The listing builds one solid part. Answer for the finished solid, in the listing's coordinates (mm). A direction names the side the tool comes from. Give positions to 0.01 mm unless a question says otherwise; leave off trailing zeros. Order: outer loops, then holes, each group sorted by start corner. A loop starts at its lowest first (then second) coordinate and runs counter-clockwise, first axis right, second up. Notation, with made-up numbers: M 33.5,77.5 L 79.5,77.5 A14 ccw 79.5,101.5 Z; hole C 20.25,29 d6. An arc over 180 degrees is marked long. Answer as a JSON object with one key per item and string values. Group by question number.
```python
from build123d import *

# Parameters (mm, degrees)
SKETCH_1_R                   = 56
EXTRUDE_1_DEPTH              = 10
SKETCH_2_R                   = 15
EXTRUDE_2_DEPTH              = 25
M20X1_5_1_D                  = 18.5
M20X1_5_1_DEPTH              = 44.5
M20X1_5_1_TIP                = 5.557960726
HOLE_WIZARD_M6_1_D           = 6.6
HOLE_WIZARD_M6_1_CSINK_D     = 13.44
HOLE_WIZARD_M6_1_CSINK_ANGLE = 90
SKETCH_12_OUTSIDE_W          = 146.442
SKETCH_12_OUTSIDE_H          = 146.442
SKETCH_12_OUTSIDE_W_2        = 136.125327254
SKETCH_12_OUTSIDE_H_2        = 80
CUT_EXTRUDE_1_DEPTH          = 25
SKETCH_13_W                  = 2
SKETCH_13_H                  = 2.5
CHAMFER_7_SIZE               = 0.5
SKETCH_14_R                  = 15
CUT_EXTRUDE_2_DEPTH          = 5


with BuildPart() as part:
    # 草图1 → 凸台-拉伸1 (new body)
    with BuildSketch(Plane(origin=(0, 0, 0), x_dir=(1, 0, 0), z_dir=(0, 1, 0))):
        with Locations(Location((0, 0, 0), (0, 0, 270))):
            Circle(SKETCH_1_R)
    extrude(amount=EXTRUDE_1_DEPTH)

    # 草图2 → 凸台-拉伸2 (add)
    with BuildSketch(Plane(origin=(0, 10, 0), x_dir=(1, 0, 0), z_dir=(0, 1, 0))):
        with Locations(Location((0, 0, 0), (0, 0, 270))):
            Circle(SKETCH_2_R)
    extrude(amount=EXTRUDE_2_DEPTH)

    # M20x1.5 螺纹孔1
    with Locations(Plane(origin=(0, 35, 0), x_dir=(1, 0, 0), z_dir=(0, 1, 0))):
        with Locations((0, 0)):
            Hole(M20X1_5_1_D / 2, depth=M20X1_5_1_DEPTH)
            with Locations((0, 0, -(M20X1_5_1_DEPTH + M20X1_5_1_TIP / 2))):  # 118° drill point
                Cone(0, M20X1_5_1_D / 2, M20X1_5_1_TIP, mode=Mode.SUBTRACT)

    # M6 六角凹锥坑螺钉的锥形沉头孔1 (through all)
    with Locations(Plane(origin=(0, 10, 0), x_dir=(1, 0, 0), z_dir=(0, 1, 0))):
        with Locations((44.346217561, -18.368804754), (-44.346217561, 18.368804754), (-44.346217561, -18.368804754), (44.346217561, 18.368804754)):
            CounterSinkHole(HOLE_WIZARD_M6_1_D / 2, HOLE_WIZARD_M6_1_CSINK_D / 2, counter_sink_angle=HOLE_WIZARD_M6_1_CSINK_ANGLE)

    # 草图12 outside → 切除-拉伸1 (cut)
    with BuildSketch(Plane(origin=(0, 10, 0), x_dir=(1, 0, 0), z_dir=(0, 1, 0))):
        Rectangle(SKETCH_12_OUTSIDE_W, SKETCH_12_OUTSIDE_H)
        Rectangle(SKETCH_12_OUTSIDE_W_2, SKETCH_12_OUTSIDE_H_2, mode=Mode.SUBTRACT)
    extrude(amount=-CUT_EXTRUDE_1_DEPTH, mode=Mode.SUBTRACT)

    # 草图13 → 切除-旋转1 (revolve, cut)
    with BuildSketch(Plane.XY, mode=Mode.PRIVATE) as cut_revolve_1_sk:
        with Locations((-14, 11.25)):
            Rectangle(SKETCH_13_W, SKETCH_13_H)
    revolve(cut_revolve_1_sk.sketch.rotate(Axis((0, -2.79729943, 0), (0, 1, 0)), 270), axis=Axis((0, -2.79729943, 0), (0, 1, 0)), mode=Mode.SUBTRACT)

    # 倒角7
    chamfer_7_edges = [part.edges().sort_by_distance(p)[0] for p in [
        (56, 0, 0),
        (56, 10, 0),
        (-56, 0, 0),
        (0, 0, -40),
        (0, 0, 40),
        (-56, 10, 0),
        (0, 10, 40),
        (0, 10, -40),
        (0, 35, -15),
    ]]
    chamfer(chamfer_7_edges, length=CHAMFER_7_SIZE)

    # 草图14 → 切除-拉伸2 (cut)
    with BuildSketch(Plane.XZ):
        with Locations(Location((0, 0, 0), (0, 0, 270))):
            Circle(SKETCH_14_R)
    extrude(amount=-CUT_EXTRUDE_2_DEPTH, mode=Mode.SUBTRACT)


solid = part.part
```
Item 1: A tool of negligible diameter and unlimited length cuts with its end or side. For faces 4 (the conical face through (-55.632, 9.865, -0.62)), 5 (the cylindrical face through (0.66, 2.465, 14.985)), 6 (the flat face through (-13.4, 12.5, 0.1)), from which of +Z, -Z, +X, -X, +Y, -Y can it reach the whole face along a straight path? Write none if from no direction.
Item 2: Consider probe 1 along Z at (x, y) = (-45, 3); probe 2 along Y at (x, z) = (-36, -26); probe 3 along Z at (x, y) = (1.5, 21). Determine where each line is inside the solid, lowest interval first. Write a range as from..to.
Item 3: Section D-D (y = 23.5) is taken. Determine the outline of the cut face in (x, z), and give its area (3 significant figures).
Item 4: Section B-B (z = 0) is taken. Determine the outline of the cut face in (x, y), and give its area (3 significant figures).
Item 5: Flat-ended cylindrical pins translate along their axes: P1, Ø6, axis at x = 7, y = 24, coming from the -Z side; P2, Ø4, axis at x = -44.35, z = -18.37, coming from the +Y side (3 decimals); P3, Ø6, axis at x = -42, y = 12, coming from the +Z side; P4, Ø8.5, axis at x = 44.35, z = -18.37, coming from the +Y side. Find the tip coordinate at first contact, or state that the pin passes through.
Item 6: Determine the mould class of faces 1 (the cylindrical face through (55.997, 4.937, 0.624)), 2 (the conical face through (41.04, 6.746, 17.328)), 3 (the flat face through (13, 0, 8)) for opening direction Z: released by +Z, released by -Z, zero draft, split by the parting line, or undercut.
Item 7: Section C-C (x = -30) is taken. Determine the outline of the cut face in (y, z).
Item 8: Section A-A (x = 0) is taken. Determine the outline of the cut face in (y, z).
Values found:
{
 "1": {"face 4": "-X, +Y", "face 5": "-Y", "face 6": "none"},
 "2": {"probe 1": "z = -33.33..-21.6, -15.13..15.13, 21.6..33.33", "probe 2": "y = 0..10", "probe 3": "z = -14.92..-9.13, 9.13..14.92"},
 "3": {"outline": "C 0,0 d30; hole C 0,0 d18.5", "area": "438 mm^2"},
 "4": {"outline": "M -56,0.5 L -55.5,0 L -15,0 L -15,5 L -9.25,5 L -9.25,35 L -14.5,35 L -15,34.5 L -15,12.5 L -13,12.5 L -13,10 L -55.5,10 L -56,9.5 Z; M 9.25,5 L 15,5 L 15,0 L 55.5,0 L 56,0.5 L 56,9.5 L 55.5,10 L 13,10 L 13,12.5 L 15,12.5 L 15,34.5 L 14.5,35 L 9.25,35 Z", "area": "1,150 mm^2"},
 "5": {"P1": "stops at z = -14.46", "P2": "passes through", "P3": "stops at z = 38.84", "P4": "stops at y = 7.53"},
 "6": {"face 1": "split by the parting line", "face 2": "undercut", "face 3": "zero draft"},
 "7": {"outline": "M 0,-39.5 L 0.5,-40 L 9.5,-40 L 10,-39.5 L 10,39.5 L 9.5,40 L 0.5,40 L 0,39.5 Z"},
 "8": {"outline": "M 0,-39.5 L 0.5,-40 L 9.5,-40 L 10,-39.5 L 10,-13 L 12.5,-13 L 12.5,-15 L 34.5,-15 L 35,-14.5 L 35,-9.25 L 5,-9.25 L 5,-15 L 0,-15 Z; M 0,15 L 5,15 L 5,9.25 L 35,9.25 L 35,14.5 L 34.5,15 L 12.5,15 L 12.5,13 L 10,13 L 10,39.5 L 9.5,40 L 0.5,40 L 0,39.5 Z"}
}
